from build123d import *

# Parameters (mm, degrees)
SKETCH_1_R               = 125
EXTRUDE_1_DEPTH          = 10
M5X0_8_1_AT_2_COUNT      = 2
M5X0_8_1_AT_2_PITCH      = 20.705523608
PATTERN_CIRCULAR_1_COUNT = 3


with BuildPart() as part:
    # 草图1 → 凸台-拉伸1 (new body)
    with BuildSketch(Plane.XY):
        Circle(SKETCH_1_R)
    extrude(amount=EXTRUDE_1_DEPTH)

    # 草图4 → M5x0.8 螺纹孔1 (revolve, cut)
    with BuildSketch(Plane(origin=(10.352761804, 38.637033052, 10), x_dir=(0, -1, 0), z_dir=(1, 0, 0))):
        Polygon((0, 0), (0, 13.6618073), (2.1, 12.4), (2.1, 0.425), (2.525, 0), align=None)
    m5x0_8_1 = revolve(axis=Axis((10.352761804, 38.637033052, 16.35), (0, 0, -1)), mode=Mode.SUBTRACT)

    # M5x0.8 螺纹孔1 at 2: M5x0.8 螺纹孔1 ×2
    with Locations(*[(-i * M5X0_8_1_AT_2_PITCH, 0, 0) for i in range(1, M5X0_8_1_AT_2_COUNT)]):
        add(m5x0_8_1, mode=Mode.SUBTRACT)

    # 阵列(圆周)1: M5x0.8 螺纹孔1 ×3 about axis
    pattern_circular_1_axis = Axis((0, 0, 0), (0, 0, 1))
    for i in range(1, PATTERN_CIRCULAR_1_COUNT):
        add(m5x0_8_1.rotate(pattern_circular_1_axis, i * 360 / PATTERN_CIRCULAR_1_COUNT), mode=Mode.SUBTRACT)

    # 阵列(圆周)1 copy 1 sketch → 阵列(圆周)1 copy 1 (revolve, cut)
    with BuildSketch(Plane(origin=(-28.284271247, -28.284271247, 10), x_dir=(0.8660254037844387, 0.4999999999999998, 0), z_dir=(-0.4999999999999998, 0.8660254037844387, 0))):
        Polygon((0, 0), (0, 13.6618073), (2.1, 12.4), (2.1, 0.425), (2.525, 0), align=None)
    revolve(axis=Axis((-28.284271247, -28.284271247, 16.35), (0, 0, -1)), mode=Mode.SUBTRACT)

    # 阵列(圆周)1 copy 2 sketch → 阵列(圆周)1 copy 2 (revolve, cut)
    with BuildSketch(Plane(origin=(38.637033052, -10.352761804, 10), x_dir=(-0.8660254037844384, 0.5000000000000004, 0), z_dir=(-0.5000000000000004, -0.8660254037844384, 0))):
        Polygon((0, 0), (0, 13.6618073), (2.1, 12.4), (2.1, 0.425), (2.525, 0), align=None)
    revolve(axis=Axis((38.637033052, -10.352761804, 16.35), (0, 0, -1)), mode=Mode.SUBTRACT)


solid = part.part
Read the model definition and answer for the solid it produces. Units are mm, in the model's axes. Give positions to 0.01 mm unless a question says otherwise; leave off trailing zeros. Loops run counter-clockwise (first coordinate to the right, second up) from the corner with the lowest first, then second, coordinate; pieces in that order, holes last. Notation, with made-up numbers: (26, 35) - (76, 35) arc R36 cw to (76, 73) - close; hole circle Ø2 at (89, 70). An arc over 180 degrees is marked (long way). Answer as CSV lines item,"result". Start each with the question number.
1) Each of these flat-tipped pins is pushed along its axis until it touches: pin 1 Ø3.5 at (x, y) = (-28.28, -28.28) entering from -Z; pin 2 Ø1.5 at (x, z) = (-88.5, 2.5) entering from +Y; pin 3 Ø6 at (y, z) = (90, 2) entering from +X; pin 4 Ø1 at (x, z) = (35.5, 1.5) entering from -Y. Where does it stop, or does it pass through?
2) Find section A-A (z = 6). Write down the section's boundary in (x, y).
3) Find section C-C (x = -108). Write down the section's boundary in (y, z).
4) Determine the mould class of faces 1 (the face through (-2, 2, 10)), 2 (the face through (-124.88, 5.5, 4.93)), 3 (the face through (-2, 2, 0)) for opening direction Z: released by +Z, released by -Z, zero draft, split by the parting line, or undercut.
5) Find section B-B (y = -63). Write down the section's boundary in (x, z).
6) Straight lines are drawn through the part: L1, parallel to X at y = 40, z = 4.25; L2, parallel to Y at x = -10, z = 1.75; L3, parallel to X at y = 39, z = 4.75. For each, find the intervals that lie inside material, in ascending order. Write a range as from..to.
Findings below:
1,pin 1,"through"
1,pin 2,"y = 89.02"
1,pin 3,"x = 89.76"
1,pin 4,"y = -120"
2,outline,"circle Ø250 at (0, 0); hole circle Ø4.2 at (-38.64, -10.35); hole circle Ø4.2 at (-28.28, -28.28); hole circle Ø4.2 at (-10.35, 38.64); hole circle Ø4.2 at (10.35, 38.64); hole circle Ø4.2 at (28.28, -28.28); hole circle Ø4.2 at (38.64, -10.35)"
3,outline,"(-62.94, 0) - (62.94, 0) - (62.94, 10) - (-62.94, 10) - close"
4,face 1,"released by +Z"
4,face 2,"zero draft"
4,face 3,"released by -Z"
5,outline,"(-107.96, 0) - (107.96, 0) - (107.96, 10) - (-107.96, 10) - close"
6,L1,"-118.43..-11.95, -8.76..8.76, 11.95..118.43"
6,L2,"-124.6..36.57, 40.71..124.6"
6,L3,"-118.76..-12.42, -8.28..8.28, 12.42..118.76"
